The model under review builds one solid part; all positions refer to its coordinate system, in mm. A direction names the side the tool comes from. Round coordinates to 2 decimals unless told otherwise and drop trailing zeros. Loops run counter-clockwise (first coordinate to the right, second up) from the corner with the lowest first, then second, coordinate; pieces in that order, holes last. Notation, with made-up numbers: M 28,61.5 L 53,61.5 A35 cw 53,98.5 Z; hole C 13,32 d9. An arc over 180 degrees is marked long. Answer as a JSON object with one key per item and string values. Group by question number.
Item 1: Consider section B-B (z = 13). Give the boundary of the cut face in (x, y).
Item 2: Insertion check: P1, Ø1.3, axis at x = 153.5, z = 12.5, coming from the +Y side; P2, Ø2, axis at y = 153, z = 17, coming from the -X side; P3, Ø12, axis at x = -125, z = 10.5, coming from the +Y side. Each pin has a flat end and moves straight along its axis. Give the tip position at first contact, or say it passes through.
Item 3: Consider section A-A (y = 0). Give the boundary of the cut face in (x, z).
Item 4: Tool access review of faces 4 (the face through (108.964, -106.692, 17.03)), 5 (the face through (35.769, -161.076, 0.74)), 6 (the face through (98.5, -123.3, 35)), 7 (the face through (-34.143, -153.755, 34.014)), 8 (the face through (12, -165, 0)): name each direction out of +Z, -Z, +X, -X, +Y, -Y from which nothing blocks a thin tool from reaching the whole face with its end or side.
Item 5: To check wall thickness, follow line 1 (Y direction, x = 0, z = 34.45); line 2 (Y direction, x = 0, z = 1); line 3 (X direction, y = 10, z = 9). State the ranges of each line that lie inside material, in increasing order.
Item 6: The part is to be moulded in two halves that separate along X. For faces 1 (the face through (-132.922, -101.921, 33.986)), 2 (the face through (142, -90, 33)), 3 (the face through (-106.692, -108.964, 17.03)), say which applies: +X half, -X half, draft (parallel to the pull), parting line (faces both ways), or undercut.
```python
from build123d import *

# Parameters (mm, degrees)
SKETCH1_R           = 175
BOSS_EXTRUDE1_DEPTH = 35
CUT_EXTRUDE1_START  = -2
SKETCH2_R           = 175
SKETCH2_R_2         = 167.5
CUT_EXTRUDE1_DEPTH  = 2
SKETCH3_R           = 157.5
CUT_EXTRUDE2_DEPTH  = 2
SKETCH4_R           = 165
CUT_EXTRUDE3_DEPTH  = 1.5
SKETCH5_R           = 152.5
CUT_EXTRUDE4_DEPTH  = 250.744369306
SKETCH7_W           = 10
SKETCH7_H           = 310
CUT_EXTRUDE6_DEPTH  = 99.5
CIRPATTERN1_COUNT   = 4
SKETCH8_OUTSIDE_W   = 2071.968
SKETCH8_OUTSIDE_H   = 2071.968
SKETCH8_OUTSIDE_R   = 172
CUT_EXTRUDE7_DEPTH  = 99.5
CUT_EXTRUDE7_DRAFT  = -83


with BuildPart() as part:
    # Sketch1 → Boss-Extrude1 (new body)
    with BuildSketch(Plane.XY):
        Circle(SKETCH1_R)
    extrude(amount=BOSS_EXTRUDE1_DEPTH)

    # Sketch2 → Cut-Extrude1 (cut)
    with BuildSketch(Plane.XY.offset(35).offset(CUT_EXTRUDE1_START)):
        Circle(SKETCH2_R)
        Circle(SKETCH2_R_2, mode=Mode.SUBTRACT)
    extrude(amount=CUT_EXTRUDE1_DEPTH, mode=Mode.SUBTRACT)

    # Sketch3 → Cut-Extrude2 (cut)
    with BuildSketch(Plane.XY.offset(35)):
        Circle(SKETCH3_R)
    extrude(amount=-CUT_EXTRUDE2_DEPTH, mode=Mode.SUBTRACT)

    # Sketch4 → Cut-Extrude3 (cut)
    with BuildSketch(Plane(origin=(0, 0, 0), x_dir=(-1, 0, 0), z_dir=(0, 0, -1))):
        Circle(SKETCH4_R)
    extrude(amount=-CUT_EXTRUDE3_DEPTH, mode=Mode.SUBTRACT)

    # Sketch5 → Cut-Extrude4 (cut, through all)
    with BuildSketch(Plane(origin=(0, 0, 1.5), x_dir=(-1, 0, 0), z_dir=(0, 0, -1))):
        Circle(SKETCH5_R)
    extrude(amount=-CUT_EXTRUDE4_DEPTH, mode=Mode.SUBTRACT)

    # Sketch7 → Cut-Extrude6 (cut)
    with BuildSketch(Plane(origin=(0, 0, 1.5), x_dir=(-1, 0, 0), z_dir=(0, 0, -1))):
        Rectangle(SKETCH7_W, SKETCH7_H)
    cut_extrude6 = extrude(amount=-CUT_EXTRUDE6_DEPTH, mode=Mode.SUBTRACT)

    # CirPattern1: Cut-Extrude6 ×4 about axis
    cirpattern1_axis = Axis((0, 0, 0), (0, 0, 1))
    for i in range(1, CIRPATTERN1_COUNT):
        add(cut_extrude6.rotate(cirpattern1_axis, i * 360 / CIRPATTERN1_COUNT), mode=Mode.SUBTRACT)


with BuildPart() as cut_extrude7_tool:
    # Sketch8 outside → Cut-Extrude7 (with draft: the straight prism first)
    with BuildSketch(Plane(origin=(0, 0, 0), x_dir=(-1, 0, 0), z_dir=(0, 0, -1))):
        Rectangle(SKETCH8_OUTSIDE_W, SKETCH8_OUTSIDE_H)
        Circle(SKETCH8_OUTSIDE_R, mode=Mode.SUBTRACT)
    extrude(amount=-CUT_EXTRUDE7_DEPTH)
    # Cut-Extrude7: the draft: its side faces are tilted about the plane it starts from
    cut_extrude7_sides = [cut_extrude7_tool.faces().sort_by_distance(p)[0] for p in [
        (0, -1035.984, 49.75),
        (-1035.984, 0, 49.75),
        (0, 1035.984, 49.75),
        (1035.984, 0, 49.75),
        (172, 0, 49.75),
    ]]
    draft(cut_extrude7_sides, Plane(origin=(0, 0, 0), x_dir=(-1, 0, 0), z_dir=(0, 0, -1)), CUT_EXTRUDE7_DRAFT)


with BuildPart() as part_1:
    add(part.part)

    # Cut-Extrude7: cut by cut_extrude7_tool
    add(cut_extrude7_tool.part, mode=Mode.SUBTRACT)


solid = part_1.part
```
Geometry results:
{
 "1": {"outline": "C 0,0 d350; hole M -155,-5 L -152.42,-5 A152.5 ccw -5,-152.42 L -5,-155 L 5,-155 L 5,-152.42 A152.5 ccw 152.42,-5 L 155,-5 L 155,5 L 152.42,5 A152.5 ccw 5,152.42 L 5,155 L -5,155 L -5,152.42 A152.5 ccw -152.42,5 L -155,5 Z"},
 "2": {"P1": "stops at y = 85.22", "P2": "stops at x = -86.72", "P3": "stops at y = 128.31"},
 "3": {"outline": "M -175,0.37 L -172,0 L -165,0 L -165,1.5 L -155,1.5 L -155,33 L -157.5,33 L -157.5,35 L -167.5,35 L -167.5,33 L -175,33 Z; M 155,1.5 L 165,1.5 L 165,0 L 172,0 L 175,0.37 L 175,33 L 167.5,33 L 167.5,35 L 157.5,35 L 157.5,33 L 155,33 Z"},
 "4": {"face 4": "+Z, -Z", "face 5": "-Z", "face 6": "+Z, +X, -X, +Y, -Y", "face 7": "+Z", "face 8": "-Z, +X, -X, +Y, -Y"},
 "5": {"line 1": "y = -167.5 to -157.5, 157.5 to 167.5", "line 2": "y = -175 to -165, 165 to 175", "line 3": "x = -174.71 to -152.17, 152.17 to 174.71"},
 "6": {"face 1": "parting line", "face 2": "draft", "face 3": "undercut"}
}
